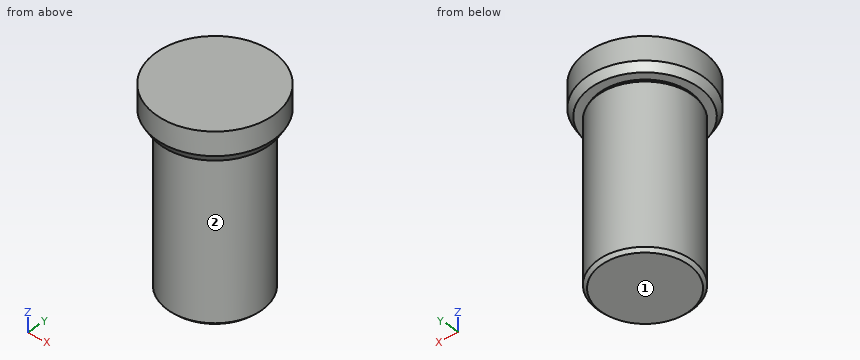
```python
from build123d import *

# Parameters (mm, degrees)
SKETCH_1_R      = 30
EXTRUDE_1_DEPTH = 105
SKETCH_2_R      = 37.5
EXTRUDE_2_DEPTH = 20
CHAMFER_2_SIZE  = 2
SKETCH_3_W      = 1
SKETCH_3_H      = 2
CHAMFER_3_SIZE  = 5
CHAMFER_3_SIZE2 = 2.886751346


with BuildPart() as part:
    # 草图1 → 凸台-拉伸1 (new body)
    with BuildSketch(Plane.XY):
        Circle(SKETCH_1_R)
    extrude(amount=EXTRUDE_1_DEPTH)

    # 草图2 → 凸台-拉伸2 (add)
    with BuildSketch(Plane.XY.offset(105)):
        Circle(SKETCH_2_R)
    extrude(amount=EXTRUDE_2_DEPTH)

    # 倒角2
    chamfer_2_edges = [part.edges().sort_by_distance(p)[0] for p in [
        (-30, 0, 0),
    ]]
    chamfer(chamfer_2_edges, length=CHAMFER_2_SIZE)

    # 草图3 → 切除-旋转1 (revolve, cut)
    with BuildSketch(Plane(origin=(0, 0, 0), x_dir=(1, 0, 0), z_dir=(0, 1, 0))):
        with Locations((29.5, -104)):
            Rectangle(SKETCH_3_W, SKETCH_3_H)
    revolve(axis=Axis((0, 0, 105), (0, 0, -1)), mode=Mode.SUBTRACT)

    # 倒角3
    chamfer_3_edges = [part.edges().sort_by_distance(p)[0] for p in [
        (-37.5, 0, 105),
    ]]
    chamfer_3_side = [part.faces().sort_by_distance(p)[0] for p in [
        (-37.5, 0, 115),
    ]]
    chamfer(chamfer_3_edges, length=CHAMFER_3_SIZE, length2=CHAMFER_3_SIZE2, reference=chamfer_3_side[0])


solid = part.part
```
Source: CAD feature listing. Evaluate the final solid. Frame: model axes, mm. Face numbers are marked on the shaded views. A direction names the side the tool comes from. Give positions to 0.01 mm unless a question says otherwise; leave off trailing zeros. Order: outer loops, then holes, each group sorted by start corner. A loop starts at its lowest first (then second) coordinate and runs counter-clockwise, first axis right, second up.
(1) Contact query for flat-ended pins moving along their axis: P1, Ø6, axis at y = 26.5, z = 104, coming from the +X side; P2, Ø1, axis at x = -24.5, z = 82.5, coming from the -Y side; P3, Ø2, axis at y = -11.5, z = 67.5, coming from the +X side. Output: stop coordinate, or through.
(2) Section query C-C (z = 27). Return the cut outline in (x, y).
(3) Access query for the marked faces 1 and 2. Directions: +Z, -Z, +X, -X, +Y, -Y. A direction counts if a zero-diameter tool reaches every point of the face in a straight line with its end or side. Return the directions, or none.
(4) Section query A-A (x = 0). Return the cut outline in (y, z).
(5) Material intervals for line 1 along Y through (x, z) = (-1, 104.5); line 2 along Y through (x, z) = (-0.5, 18); line 3 along Z through (x, y) = (-25.5, -23), sorted ascending.
Outcome:
1. P1: stops at x = 25.49
1. P2: stops at y = -18
1. P3: stops at x = 28.1
2. outline: circle Ø60 at (0, 0)
3. face 1: -Z, +X, -X, +Y, -Y
3. face 2: -Z
4. outline: (-37.5, 110) - (-34.61, 105) - (-29, 105) - (-29, 103) - (-30, 103) - (-30, 2) - (-28, 0) - (28, 0) - (30, 2) - (30, 103) - (29, 103) - (29, 105) - (34.61, 105) - (37.5, 110) - (37.5, 125) - (-37.5, 125) - close
5. line 1: y = -28.98 to 28.98
5. line 2: y = -30 to 30
5. line 3: z = 105 to 125
